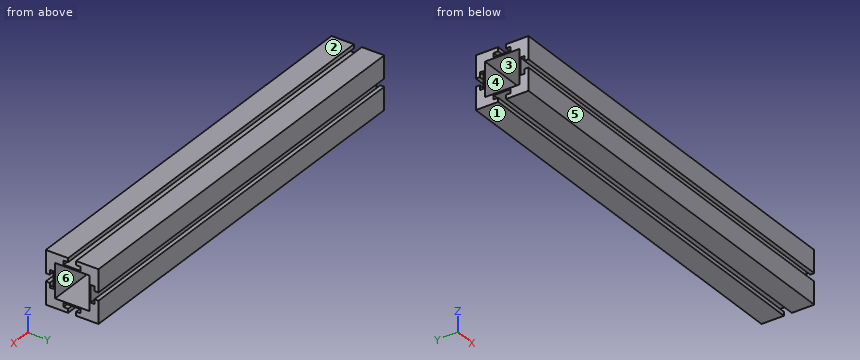
from build123d import *

# Parameters (mm, degrees)
SKETCH1_W           = 26
SKETCH1_H           = 26
BOSS_EXTRUDE1_DEPTH = 310


with BuildPart() as part:
    # Sketch1 → Boss-Extrude1 (new body)
    with BuildSketch(Plane(origin=(0, 0, 0), x_dir=(0, 0, -1), z_dir=(1, 0, 0))):
        Polygon((-20, -20), (-3, -20), (-3, -17), (-6.5, -17), (-6.5, -14), (6.5, -14), (6.5, -17), (3, -17), (3, -20), (20, -20), (20, -3), (17, -3), (17, -6.5), (14, -6.5), (14, 6.5), (17, 6.5), (17, 3), (20, 3), (20, 20), (3, 20), (3, 17), (6.5, 17), (6.5, 14), (-6.5, 14), (-6.5, 17), (-3, 17), (-3, 20), (-20, 20), (-20, 3), (-17, 3), (-17, 6.5), (-14, 6.5), (-14, -6.5), (-17, -6.5), (-17, -3), (-20, -3), align=None)
        Rectangle(SKETCH1_W, SKETCH1_H, mode=Mode.SUBTRACT)
    extrude(amount=BOSS_EXTRUDE1_DEPTH)


solid = part.part
The listing builds one solid part. Answer for the finished solid, in the listing's coordinates (mm). Face numbers are marked on the shaded views. A direction names the side the tool comes from. Coordinates: 2 decimals unless noted, no trailing zeros. Order: outer loops, then holes, each group sorted by start corner. A loop starts at its lowest first (then second) coordinate and runs counter-clockwise, first axis right, second up.
Q1. A cutting plane is placed at A-A, the plane z = 0. Write down the section's boundary in (x, y), and give its area (3 significant figures).
Q2. For a pull along Z with two mould halves and no side action, classify the marked faces 1, 2, 3 and 4 as pulls with the +Z half, pulls with the -Z half, needs draft (parallel to the pull), parting line crosses it, or undercut.
Q3. Given P1, Ø5, axis at x = 94.5, z = -1, coming from the +Y side, flat-ended and moving along its own axis, determine where the tip first touches the part or whether it passes through.
Q4. Consider line 1 (Z direction, x = 49, y = 3.5); line 2 (Z direction, x = 83.5, y = -15.5). Determine where each line is inside the solid, lowest interval first.
Q5. Which of the six approach directions +Z, -Z, +X, -X, +Y, -Y give full straight-line access (tool end or side, diameter ignored) to the marked faces 5 and 6?
Answers follow:
1. outline: (0, -14) - (310, -14) - (310, -13) - (0, -13) - close; (0, 13) - (310, 13) - (310, 14) - (0, 14) - close
1. area: 620 mm2
2. face 1: pulls with the -Z half
2. face 2: pulls with the +Z half
2. face 3: undercut
2. face 4: undercut
3. P1: stops at y = 20
4. line 1: z = -20 to -17, -14 to -13, 13 to 14, 17 to 20
4. line 2: z = -20 to -6.5, 6.5 to 20
5. face 5: +Z, -Z, +X, -X, -Y
5. face 6: +X, -X
